Read the model definition and answer for the solid it produces. Units are mm, in the model's axes. Face numbers are marked on the shaded views. A direction names the side the tool comes from. Coordinates: 2 decimals unless noted, no trailing zeros. Write each loop counter-clockwise with the first axis right and the second up, starting at its lowest first coordinate (ties: lowest second). Pieces come first, ordered by that corner, then holes. Notation, with made-up numbers: (18.5, 81.5) - (62.5, 81.5) arc R19 ccw to (62.5, 87.5) - close; hole circle Ø5 at (-25.5, -6). An arc over 180 degrees is marked (long way). Use a Markdown table: item, result.
from build123d import *

# Parameters (mm, degrees)
SKETCH1_W           = 65
SKETCH1_H           = 65
BOSS_EXTRUDE1_DEPTH = 10
SKETCH2_R           = 20
BOSS_EXTRUDE2_DEPTH = 50.8
FILLET1_R           = 20
SKETCH3_R           = 1.5
CUT_EXTRUDE1_DEPTH  = 5


with BuildPart() as part:
    # Sketch1 → Boss-Extrude1 (new body)
    with BuildSketch(Plane(origin=(0, 0, 0), x_dir=(1, 0, 0), z_dir=(0, 1, 0))):
        Rectangle(SKETCH1_W, SKETCH1_H)
    extrude(amount=BOSS_EXTRUDE1_DEPTH)

    # Sketch2 → Boss-Extrude2 (add)
    with BuildSketch(Plane(origin=(0, 10, 0), x_dir=(1, 0, 0), z_dir=(0, 1, 0))):
        with Locations(Location((0, 0, 0), (0, 0, 270))):
            Circle(SKETCH2_R)
    extrude(amount=BOSS_EXTRUDE2_DEPTH)

    # Fillet1
    fillet1_edges = [part.edges().sort_by_distance(p)[0] for p in [
        (0, 60.8, -20),
    ]]
    fillet(fillet1_edges, radius=FILLET1_R)

    # Sketch3 → Cut-Extrude1 (cut)
    with BuildSketch(Plane.XZ):
        with Locations(Location((24, 18, 0), (0, 0, 270))):
            Circle(SKETCH3_R)
        with Locations(Location((-24, 18, 0), (0, 0, 270))):
            Circle(SKETCH3_R)
        with Locations(Location((-24, -18, 0), (0, 0, 270))):
            Circle(SKETCH3_R)
        with Locations(Location((24, -18, 0), (0, 0, 270))):
            Circle(SKETCH3_R)
    extrude(amount=-CUT_EXTRUDE1_DEPTH, mode=Mode.SUBTRACT)


solid = part.part
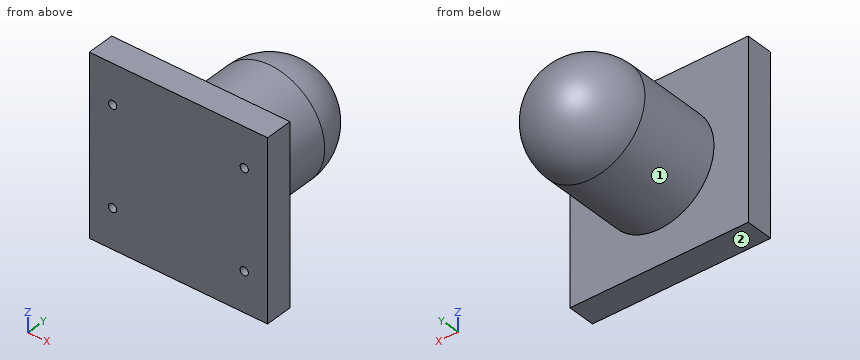
(1) A cutting plane is placed at A-A, the plane x = 0. Write down the section's boundary in (y, z).
Report:
| item | result |
|---|---|
| outline | (0, -32.5) - (10, -32.5) - (10, -20) - (40.8, -20) arc R20 ccw to (40.8, 20) - (10, 20) - (10, 32.5) - (0, 32.5) - close |
(2) For the marked faces 1 and 2, determine the directions among +Z, -Z, +X, -X, +Y, -Y from which every point of the face is accessible in a straight line to the end or side of a thin tool.
Report:
| item | result |
|---|---|
| face 1 | +Y |
| face 2 | -Z, +X, -X, +Y, -Y |
(3) A cutting plane is placed at C-C, the plane z = 18. Write down the section's boundary in (x, y).
Report:
| item | result |
|---|---|
| outline | (-32.5, 0) - (-25.5, 0) - (-25.5, 5) - (-22.5, 5) - (-22.5, 0) - (22.5, 0) - (22.5, 5) - (25.5, 5) - (25.5, 0) - (32.5, 0) - (32.5, 10) - (8.72, 10) - (8.72, 40.8) arc R8.72 ccw to (-8.72, 40.8) - (-8.72, 10) - (-32.5, 10) - close |
(4) A cutting plane is placed at D-D, the plane y = 35. Write down the section's boundary in (x, z).
Report:
| item | result |
|---|---|
| outline | circle Ø40 at (0, 0) |
(5) A cutting plane is placed at B-B, the plane x = -24. Write down the section's boundary in (y, z).
Report:
| item | result |
|---|---|
| outline | (0, -32.5) - (10, -32.5) - (10, 32.5) - (0, 32.5) - (0, 19.5) - (5, 19.5) - (5, 16.5) - (0, 16.5) - (0, -16.5) - (5, -16.5) - (5, -19.5) - (0, -19.5) - close |
(6) Each of these flat-tipped pins is pushed along its axis until it touches: P1, Ø2, axis at x = -7, y = 13.5, coming from the -Z side; P2, Ø4, axis at y = 34.5, z = -20, coming from the -X side; P3, Ø6, axis at x = -2.5, y = 52.5, coming from the +Z side. Where does it stop, or does it pass through?
Report:
| item | result |
|---|---|
| P1 | stops at z = -19.08 |
| P2 | stops at x = -8.72 |
| P3 | stops at z = 17.88 |
(7) Straight lines are drawn through the part: L1, parallel to X at y = 3.3, z = -18; L2, parallel to Y at x = -28, z = 6; L3, parallel to X at y = 31, z = 4. For each, find the intervals that lie inside material, in ascending order.
Report:
| item | result |
|---|---|
| L1 | x = -32.5 to -25.5, -22.5 to 22.5, 25.5 to 32.5 |
| L2 | y = 0 to 10 |
| L3 | x = -19.6 to 19.6 |
